Here's how the part is built. I have some questions about the finished solid (model axes, mm). Face numbers are marked on the shaded views. Coordinates: 2 decimals unless noted, no trailing zeros. Write each loop counter-clockwise with the first axis right and the second up, starting at its lowest first coordinate (ties: lowest second). Pieces come first, ordered by that corner, then holes.
Item 1: If we mould it in two halves opening along Z, with no side actions, what happens to the marked faces 1 and 2? For each: pulls with the +Z half, pulls with the -Z half, needs draft (parallel to the pull), parting line crosses it, or undercut.
Item 2: I'm going to push flat-ended pins straight in: P1, Ø4, axis at x = -37, z = -37, coming from the +Y side; P2, Ø6, axis at y = 6.5, z = 124.5, coming from the +X side; P3, Ø1.5, axis at y = 9, z = -33.5, coming from the +X side. Where does each tip first touch, or does it pass through?
Item 3: I want a section at B-B (x = 0). Please give me the cut outline in (y, z), and give its area (3 significant figures).
Item 4: I want a section at C-C (x = -80). Please give me the cut outline in (y, z), and give its area (3 significant figures).
Item 5: Please list where these lines run through material, in increasing order: line 1 (X direction, y = 11.5, z = 0); line 2 (Z direction, x = -78, y = 6); line 3 (X direction, y = 3.5, z = 5).
Item 6: I want a section at A-A (z = 0). Please give me the cut outline in (x, y).
Item 7: I want a section at D-D (x = 160). Please give me the cut outline in (y, z), and give its area (3 significant figures).
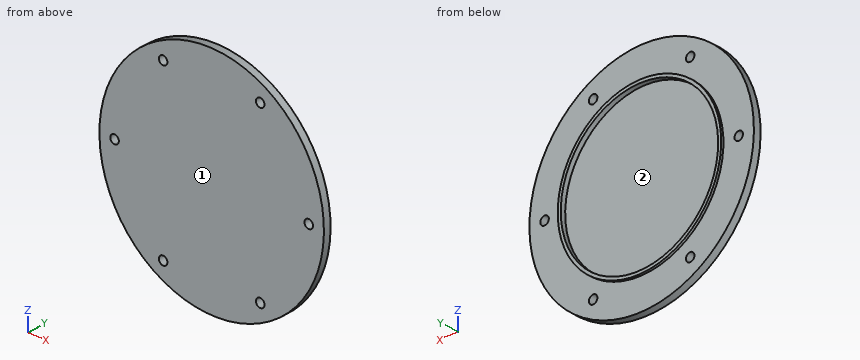
from build123d import *

# Parameters (mm, degrees)
SKETCH1_R           = 185
BOSS_EXTRUDE1_DEPTH = 12
SKETCH2_R           = 129.75
CUT_EXTRUDE1_DEPTH  = 4
BOSS_EXTRUDE2_START = 4
SKETCH3_R           = 134.75
SKETCH3_R_2         = 129.75
BOSS_EXTRUDE2_DEPTH = 4
SKETCH5_R           = 7
CUT_EXTRUDE3_DEPTH  = 262.90456277
CIRPATTERN2_COUNT   = 6


with BuildPart() as part:
    # Sketch1 → Boss-Extrude1 (new body)
    with BuildSketch(Plane(origin=(0, 0, 0), x_dir=(1, 0, 0), z_dir=(0, 1, 0))):
        with Locations(Location((0, 0, 0), (0, 0, 270))):
            Circle(SKETCH1_R)
    extrude(amount=BOSS_EXTRUDE1_DEPTH)

    # Sketch2 → Cut-Extrude1 (cut)
    with BuildSketch(Plane(origin=(0, 12, 0), x_dir=(1, 0, 0), z_dir=(0, 1, 0))):
        with Locations(Location((0, 0, 0), (0, 0, 270))):
            Circle(SKETCH2_R)
    extrude(amount=-CUT_EXTRUDE1_DEPTH, mode=Mode.SUBTRACT)

    # Sketch3 → Boss-Extrude2 (add)
    with BuildSketch(Plane(origin=(0, 12, 0), x_dir=(1, 0, 0), z_dir=(0, 1, 0)).offset(BOSS_EXTRUDE2_START)):
        with Locations(Location((0, 0, 0), (0, 0, 270))):
            Circle(SKETCH3_R)
        with Locations(Location((0, 0, 0), (0, 0, 270))):
            Circle(SKETCH3_R_2, mode=Mode.SUBTRACT)
    extrude(amount=-BOSS_EXTRUDE2_DEPTH)

    # Sketch5 → Cut-Extrude3 (cut, through all)
    with BuildSketch(Plane(origin=(0, 12, 0), x_dir=(1, 0, 0), z_dir=(0, 1, 0))):
        with Locations(Location((160, 0, 0), (0, 0, 270))):
            Circle(SKETCH5_R)
    cut_extrude3 = extrude(amount=-CUT_EXTRUDE3_DEPTH, mode=Mode.SUBTRACT)

    # CirPattern2: Cut-Extrude3 ×6 about axis
    cirpattern2_axis = Axis((0, 0, 0), (0, 1, 0))
    for i in range(1, CIRPATTERN2_COUNT):
        add(cut_extrude3.rotate(cirpattern2_axis, i * 360 / CIRPATTERN2_COUNT), mode=Mode.SUBTRACT)


solid = part.part
Answer:
1. face 1: needs draft
1. face 2: undercut
2. P1: stops at y = 8
2. P2: stops at x = 139.51
2. P3: stops at x = 182.08
3. outline: (0, -185) - (12, -185) - (12, -134.75) - (16, -134.75) - (16, -129.75) - (8, -129.75) - (8, 129.75) - (16, 129.75) - (16, 134.75) - (12, 134.75) - (12, 185) - (0, 185) - close
3. area: 3,440 mm2
4. outline: (0, -166.81) - (12, -166.81) - (12, -145.56) - (0, -145.56) - close; (0, -131.56) - (12, -131.56) - (12, -108.43) - (16, -108.43) - (16, -102.15) - (8, -102.15) - (8, 102.15) - (16, 102.15) - (16, 108.43) - (12, 108.43) - (12, 131.56) - (0, 131.56) - close; (0, 145.56) - (12, 145.56) - (12, 166.81) - (0, 166.81) - close
4. area: 2,900 mm2
5. line 1: x = -185 to -167, -153 to -129.75, 129.75 to 153, 167 to 185
5. line 2: z = -167.75 to -145.27, -131.86 to 131.86, 145.27 to 167.75
5. line 3: x = -184.93 to -164.9, -155.1 to 155.1, 164.9 to 184.93
6. outline: (-185, 0) - (-167, 0) - (-167, 12) - (-185, 12) - close; (-153, 0) - (153, 0) - (153, 12) - (134.75, 12) - (134.75, 16) - (129.75, 16) - (129.75, 8) - (-129.75, 8) - (-129.75, 16) - (-134.75, 16) - (-134.75, 12) - (-153, 12) - close; (167, 0) - (185, 0) - (185, 12) - (167, 12) - close
7. outline: (0, -92.87) - (12, -92.87) - (12, -7) - (0, -7) - close; (0, 7) - (12, 7) - (12, 92.87) - (0, 92.87) - close
7. area: 2,060 mm2
